```python
from build123d import *
from build123d.topology import SkipClean

# Parameters (mm, degrees)
SKETCH1_R           = 25
BOSS_EXTRUDE1_DEPTH = 1.5
BOSS_EXTRUDE2_DEPTH = 8
CUT_EXTRUDE2_DEPTH  = 8
SKETCH4_R           = 15
BOSS_EXTRUDE3_DEPTH = 8.5
BOSS_EXTRUDE4_DEPTH = 4
CUT_EXTRUDE3_DEPTH  = 42.809799474


with BuildPart() as part:
    # Sketch1 → Boss-Extrude1 (new, symmetric)
    with BuildSketch(Plane.XY):
        Circle(SKETCH1_R)
    extrude(amount=BOSS_EXTRUDE1_DEPTH, both=True)

    # Sketch2 → Boss-Extrude2 (add)
    with SkipClean():  # the faces are left unmerged after this step: merging them gives an invalid solid
        with BuildSketch(Plane(origin=(0, 0, -1.5), x_dir=(-1, 0, 0), z_dir=(0, 0, -1))):
            with BuildLine():
                Line((24.840821943, 2.816658516), (-24.840821943, 2.816658516))
                ThreePointArc((-24.840821943, 2.816658516), (-25, 0), (-24.840821943, -2.816658516))
                Line((-24.840821943, -2.816658516), (24.840821943, -2.816658516))
                ThreePointArc((24.840821943, -2.816658516), (24.960173763, -1.410576376), (25, 0))
                ThreePointArc((25, 0), (24.960173763, 1.410576376), (24.840821943, 2.816658516))
            make_face()
        extrude(amount=BOSS_EXTRUDE2_DEPTH)

    # Sketch3 → Cut-Extrude2 (cut)
    with BuildSketch(Plane(origin=(0, 2.816658516, 0), x_dir=(1, 0, 0), z_dir=(0, 1, 0))):
        Polygon((-29.660487574, 11.299873817), (-29.660487574, 1.5), (-24.840821943, 1.5), (-24.840821943, 9.5), (24.840821943, 9.5), (24.840821943, 1.5), (29.900960726, 1.5), (29.900960726, 11.299873817), align=None)
        with BuildLine():
            ThreePointArc((-24.840821943, 1.5), (0, 8.954423408), (24.840821943, 1.5))
            Line((24.840821943, 1.5), (24.840821943, 9.5))
            Line((24.840821943, 9.5), (-24.840821943, 9.5))
            Line((-24.840821943, 9.5), (-24.840821943, 1.5))
        make_face()
    extrude(amount=-CUT_EXTRUDE2_DEPTH, mode=Mode.SUBTRACT)

    # Sketch4 → Boss-Extrude3 (add)
    with BuildSketch(Plane.XY.offset(1.5)):
        Circle(SKETCH4_R)
    extrude(amount=BOSS_EXTRUDE3_DEPTH)

    # Sketch5 → Boss-Extrude4 (add)
    with BuildSketch(Plane.XY.offset(10)):
        with BuildLine():
            Line((-5.44764904, 17.730849129), (-5.44764904, 4.943959841))
            Line((-5.44764904, 4.943959841), (5.44764904, 4.943959841))
            Line((5.44764904, 4.943959841), (5.44764904, 17.730849129))
            ThreePointArc((5.44764904, 17.730849129), (0, 23.17849817), (-5.44764904, 17.730849129))
        make_face()
        with BuildLine():
            Line((-5.44764904, -17.730849129), (-5.44764904, -4.943959841))
            Line((-5.44764904, -4.943959841), (5.44764904, -4.943959841))
            Line((5.44764904, -4.943959841), (5.44764904, -17.730849129))
            ThreePointArc((5.44764904, -17.730849129), (0, -23.17849817), (-5.44764904, -17.730849129))
        make_face()
    extrude(amount=BOSS_EXTRUDE4_DEPTH)

    # Sketch7 → Cut-Extrude3 (cut, through all)
    with BuildSketch(Plane.ZY.offset(5.44764904)):
        Polygon((10, 23.17849817), (14, 4.943959841), (14, 23.17849817), align=None)
        Polygon((14, -23.17849817), (10, -4.943959841), (14, -4.943959841), align=None)
    extrude(amount=-CUT_EXTRUDE3_DEPTH, mode=Mode.SUBTRACT)


solid = part.part
```
Read the model definition and answer for the solid it produces. Units are mm, in the model's axes. A direction names the side the tool comes from. Give positions to 0.01 mm unless a question says otherwise; leave off trailing zeros. Write each loop counter-clockwise with the first axis right and the second up, starting at its lowest first coordinate (ties: lowest second). Pieces come first, ordered by that corner, then holes. Notation, with made-up numbers: (0.5, -8) -> (53.5, -8) arc R9 ccw to (53.5, -3) -> close; hole circle Ø10 at (81.25, 77). An arc over 180 degrees is marked (long way). Answer in a Markdown table with one row per item.
1) A tool of negligible diameter and unlimited length cuts with its end or side. For faces 5 (the cylindrical face through (0.12, -23.177, 11.972)), 6 (the cylindrical face through (4.96, 19.98, 10.32)), 7 (the flat face through (-5.448, 10, 12)), 8 (the flat face through (0, 4.944, 12)), from which of +Z, -Z, +X, -X, +Y, -Y can it reach the whole face along a straight path? Write none if from no direction.
Results list:
| item | result |
|---|---|
| face 5 | +Z, -Y |
| face 6 | +Z, +X, +Y |
| face 7 | +Z, -X, +Y, -Y |
| face 8 | +Z, +X, -X |
2) Straight lines are drawn through the part: line 1 (Y direction, x = 14.5, z = -4); line 2 (Z direction, x = 12, y = 13); line 3 (X direction, y = 16, z = 10.25). For each, find the intervals that lie inside material, in ascending order. Write a range as [from, to].
Results list:
| item | result |
|---|---|
| line 1 | [-2.82, 2.82] |
| line 2 | [-1.5, 1.5] |
| line 3 | [-5.45, 5.45] |
3) Determine the mould class of faces 1 (the flat face through (0, -11, -1.5)), 2 (the flat face through (0, -19, 10)), 3 (the cylindrical face through (-14.985, 0.66, 5.69)), 4 (the flat face through (0, 2.817, -4)) for opening direction Z: released by +Z, released by -Z, zero draft, split by the parting line, or undercut.
Results list:
| item | result |
|---|---|
| face 1 | released by -Z |
| face 2 | undercut |
| face 3 | undercut |
| face 4 | zero draft |
4) Section A-A on y = 20.5 is taken. Give the vertices of the cut face in (x, z), plus the area to 3 significant figures.
Results list:
| item | result |
|---|---|
| outline | (-14.31, -1.5) -> (14.31, -1.5) -> (14.31, 1.5) -> (-14.31, 1.5) -> close; (-4.69, 10) -> (4.69, 10) -> (4.69, 10.59) -> (-4.69, 10.59) -> close |
| area | 91.4 mm^2 |
5) Section B-B on y = 0 is taken. Give the vertices of the cut face in (x, z), plus the area to 3 significant figures.
Results list:
| item | result |
|---|---|
| outline | (-25, -1.5) -> (-24.84, -1.5) arc R45.12 ccw to (24.84, -1.5) -> (25, -1.5) -> (25, 1.5) -> (15, 1.5) -> (15, 10) -> (-15, 10) -> (-15, 1.5) -> (-25, 1.5) -> close |
| area | 656 mm^2 |
6) Section C-C on x = -19 is taken. Give the vertices of the cut face in (y, z), plus the area to 3 significant figures.
Results list:
| item | result |
|---|---|
| outline | (-16.25, -1.5) -> (-2.82, -1.5) -> (-2.82, -4.76) -> (2.82, -4.76) -> (2.82, -1.5) -> (16.25, -1.5) -> (16.25, 1.5) -> (-16.25, 1.5) -> close |
| area | 116 mm^2 |
7) Section D-D on z = 2.25 is taken. Give the vertices of the cut face in (x, y).
Results list:
| item | result |
|---|---|
| outline | circle Ø30 at (0, 0) |
8) Each of these flat-tipped pins is pushed along its axis until it touches: pin 1 Ø8 at (x, z) = (-11.5, -6) entering from +Y; pin 2 Ø3 at (x, y) = (-14, 0) entering from -Z; pin 3 Ø8 at (x, z) = (8.5, -4) entering from -Y. Where does it stop, or does it pass through?
Results list:
| item | result |
|---|---|
| pin 1 | y = 2.82 |
| pin 2 | z = -7.19 |
| pin 3 | y = -24.41 |
